```python
from build123d import *

# Parameters (mm, degrees)
CHAMFER1_SIZE      = 3
CHAMFER2_SIZE      = 0.762
FILLET1_R          = 3.175
SKETCH2_R          = 11.3157
CUT_EXTRUDE1_DEPTH = 28.702


with BuildPart() as part:
    # Sketch1 → Revolve1 (revolve)
    with BuildSketch(Plane.XY, mode=Mode.PRIVATE) as revolve1_sk:
        Polygon((137.3251, 95.2119), (-137.3251, 95.2119), (-137.3251, 77.0001), (-153.548479685, 77.0001), (-156.3751, 78.63205), (-451.6501, 78.63205), (-451.6501, 34.925), (-454.9521, 34.925), (-454.9521, 0), (454.9521, 0), (454.9521, 34.925), (451.6501, 34.925), (451.6501, 78.63205), (156.3751, 78.63205), (153.548479685, 77.0001), (137.3251, 77.0001), align=None)
    revolve(revolve1_sk.sketch.rotate(Axis((-454.9521, 0, 0), (1, 0, 0)), 180), axis=Axis((-454.9521, 0, 0), (1, 0, 0)))

    # Chamfer1
    chamfer1_edges = [part.edges().sort_by_distance(p)[0] for p in [
        (-451.6501, 78.63205, 0),
        (451.6501, 78.63205, 0),
    ]]
    chamfer(chamfer1_edges, length=CHAMFER1_SIZE)

    # Chamfer2
    chamfer2_edges = [part.edges().sort_by_distance(p)[0] for p in [
        (137.3251, 95.2119, 0),
        (-137.3251, 95.2119, 0),
    ]]
    chamfer(chamfer2_edges, length=CHAMFER2_SIZE)

    # Fillet1
    fillet1_edges = [part.edges().sort_by_distance(p)[0] for p in [
        (-137.3251, 77.0001, 0),
        (-153.548479685, 77.0001, 0),
        (153.548479685, 77.0001, 0),
        (137.3251, 77.0001, 0),
    ]]
    fillet(fillet1_edges, radius=FILLET1_R)

    # Sketch2 → Cut-Extrude1 (cut)
    with BuildSketch(Plane(origin=(0, 0, -95.2119), x_dir=(0, -1, 0), z_dir=(0, 0, -1))):
        with Locations(Location((0, 0, 0), (0, 0, 180))):
            Circle(SKETCH2_R)
    extrude(amount=-CUT_EXTRUDE1_DEPTH, mode=Mode.SUBTRACT)


solid = part.part
```
Geometry: final body of the model. Coordinates: model frame, mm. A direction names the side the tool comes from. Round coordinates to 2 decimals unless told otherwise and drop trailing zeros. Order: outer loops, then holes, each group sorted by start corner. A loop starts at its lowest first (then second) coordinate and runs counter-clockwise, first axis right, second up. Notation, with made-up numbers: (77.5, -34) -> (83.5, -34) arc R24 cw to (83.5, -7) -> close; hole circle Ø3 at (71, 13). An arc over 180 degrees is marked (long way). Use one line per item in the form item = value.
(1) Draft query along Y for faces 1 (the face through (-451.65, -33, 16)), 2 (the face through (0, 0, -66.51)), 3 (the face through (146.514, -35.531, 68.312)). Return one class per face: pulls with the +Y half, pulls with the -Y half, needs draft (parallel to the pull), parting line crosses it, or undercut.
Results list:
face_1 = needs draft
face_2 = undercut
face_3 = parting line crosses it
(2) Ray query, probe 1 along X at (y, z) = (-1.5, -72.5); probe 2 along X at (y, z) = (0, -72); probe 3 along X at (y, z) = (-56, -55). Return the intervals inside material, ascending. Write a range as [from, to].
Results list:
probe_1 = [-451.65, -11.22], [11.22, 451.65]
probe_2 = [-451.65, -11.32], [11.32, 451.65]
probe_3 = [-448.79, -156.13], [-137.81, 137.81], [156.13, 448.79]
(3) Access query for faces 4 (the face through (137.325, -42, 70)), 5 (the face through (3.399, 10.793, -81.062)), 6 (the face through (-304.56, -75, -23.62)). Directions: +Z, -Z, +X, -X, +Y, -Y. A direction counts if a zero-diameter tool reaches every point of the face in a straight line with its end or side. Return the directions, or none.
Results list:
face_4 = +X
face_5 = -Z
face_6 = -X
(4) Section A-A on x = -21. Return loops of the section in (y, z), and give its area (3 significant figures).
Results list:
outline = circle Ø190.42 at (0, 0)
area = 28,500 mm^2
(5) First-contact query: pin 1 Ø4 at (x, y) = (-61, 46.5) entering from -Z; pin 2 Ø10 at (x, z) = (61, -61) entering from +Y; pin 3 Ø4 at (y, z) = (-55, 35.5) entering from -X. Flat tips, straight axial feed; report the tip coordinate or a pass-through.
Results list:
pin_1 = -84.17
pin_2 = 77
pin_3 = -451.65
(6) Section B-B on x = -187. Return loops of the section in (y, z), and give its area (3 significant figures).
Results list:
outline = circle Ø157.26 at (0, 0)
area = 19,400 mm^2
